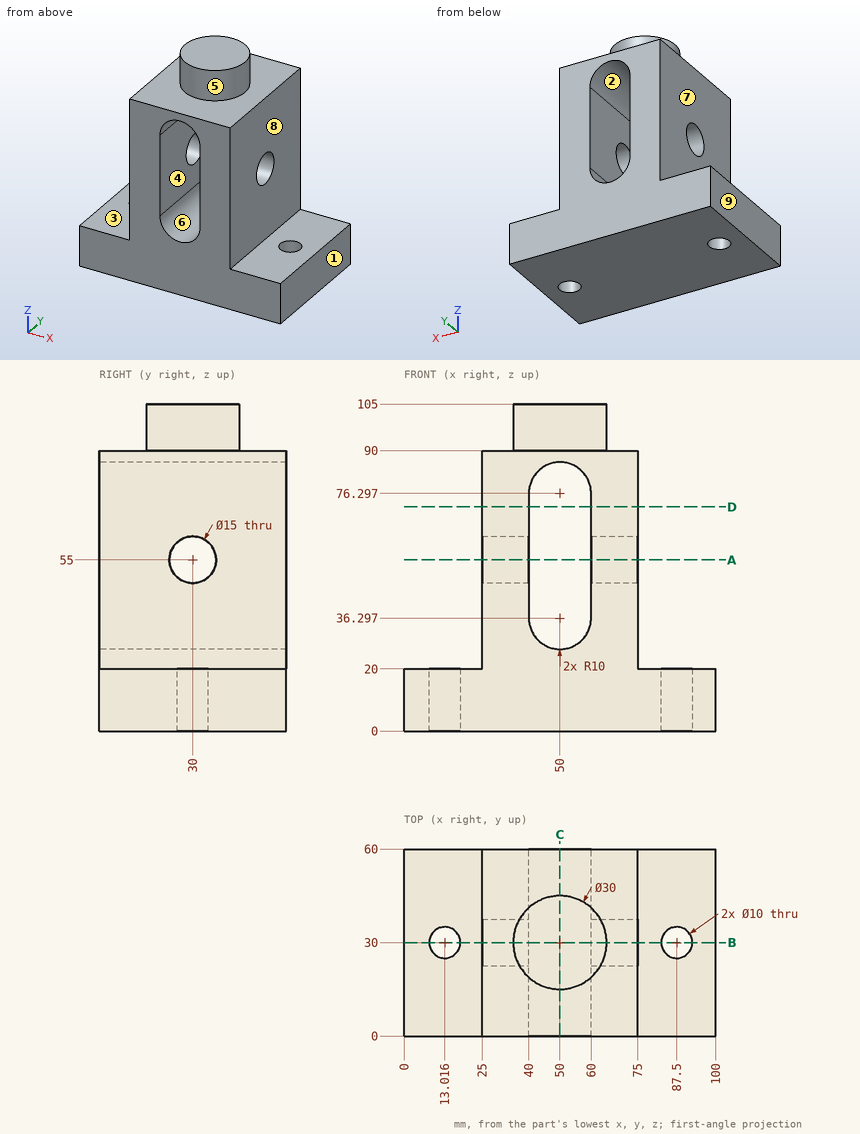
Verification items for this drawing (mm, ordinates from the low corner). A direction names the side the tool comes from. Give positions to 0.01 mm unless a question says otherwise; leave off trailing zeros. Loops run counter-clockwise (first coordinate to the right, second up) from the corner with the lowest first, then second, coordinate; pieces in that order, holes last. Notation, with made-up numbers: M 84,58 L 102,58 A24 ccw 102,84 Z; hole C -5.5,78.5 d9. An arc over 180 degrees is marked long. Answer as a JSON object with one key per item and string values. Group by question number.
Item 1: Gauge pin test, flat ends, axial feed: pin 1 (1.5 mm diameter, centred on y = 19, z = 79, fed in from +X); pin 2 (10 mm diameter, centred on y = 6.5, z = 79, fed in from -X); pin 3 (12.5 mm diameter, centred on x = 18.5, y = 36.5, fed in from +Z). Record the tip position at first contact, or that the pin passes through.
Item 2: Material ranges on L1, parallel to X at y = 4.5, z = 47.5; L2, parallel to Y at x = 63.5, z = 55; L3, parallel to X at y = 27.5, z = 12 (1 decimal), recorded low to high.
Item 3: Sectioned sample at C-C on x = 50. Record the boundary of the cut face in (y, z).
Item 4: Sectioned sample at A-A on z = 55. Record the boundary of the cut face in (x, y).
Item 5: Mould release check, pull along Z, two halves, no side actions. Record for the marked faces 1, 2, 3 and 4: pulls with the +Z half, pulls with the -Z half, needs draft (parallel to the pull), parting line crosses it, or undercut.
Item 6: Sectioned sample at D-D on z = 72. Record the boundary of the cut face in (x, y), plus the area to 3 significant figures.
Item 7: Access from +Z, -Z, +X, -X, +Y, -Y to the whole of each face (thin tool, end or side, straight path). Record for the marked faces 5, 6, 7, 8 and 9.
Item 8: Sectioned sample at B-B on y = 30. Give the number of separate pieces and of enclosed holes in the cut face, plus the area to 3 significant figures.
Findings below:
{
 "1": {"pin 1": "x = 75", "pin 2": "x = 25", "pin 3": "z = 20"},
 "2": {"L1": "25 to 40, 60 to 75", "L2": "0 to 22.5, 37.5 to 60", "L3": "0 to 8.7, 17.3 to 83.2, 91.8 to 100"},
 "3": {"outline": "M 0,0 L 60,0 L 60,26.3 L 0,26.3 Z; M 0,86.3 L 60,86.3 L 60,90 L 45,90 L 45,105 L 15,105 L 15,90 L 0,90 Z"},
 "4": {"outline": "M 25,0 L 40,0 L 40,22.5 L 25,22.5 Z; M 25,37.5 L 40,37.5 L 40,60 L 25,60 Z; M 60,0 L 75,0 L 75,22.5 L 60,22.5 Z; M 60,37.5 L 75,37.5 L 75,60 L 60,60 Z"},
 "5": {"face 1": "needs draft", "face 2": "undercut", "face 3": "pulls with the +Z half", "face 4": "undercut"},
 "6": {"outline": "M 25,0 L 40,0 L 40,60 L 25,60 Z; M 60,0 L 75,0 L 75,60 L 60,60 Z", "area": "1,800 mm2"},
 "7": {"face 5": "+Z", "face 6": "+Y, -Y", "face 7": "+Z, -X, +Y, -Y", "face 8": "+Z, +X, +Y, -Y", "face 9": "+Z, -Z, -X, +Y, -Y"},
 "8": {"separate pieces": "4", "enclosed holes": "0", "area": "3,990 mm2"}
}
